Geometry check sheet. Reference: drawing and pictorial views, mm from the part's lowest x, y, z. A direction names the side the tool comes from. Give positions to 0.01 mm unless a question says otherwise; leave off trailing zeros. Loops run counter-clockwise (first coordinate to the right, second up) from the corner with the lowest first, then second, coordinate; pieces in that order, holes last. Notation, with made-up numbers: (-24, 6.5) -> (5, 6.5) arc R22 ccw to (5, 23.5) -> close; hole circle Ø6 at (66, 88). An arc over 180 degrees is marked (long way). One line per item, written item: value. Start each with the question number.
(1) Tool access check on the marked faces 1, 2 and 3. Record the directions out of +Z, -Z, +X, -X, +Y, -Y that give a thin tool (end or side, any length) a straight path to the whole face; none if there is none.
(2) Sectioned sample at C-C, the plane z = 16.5. Record the cut outline in (x, y) (1 decimal).
(3) Scan lines: line 1 along Y through (x, z) = (4, 8.75); line 2 along X through (y, z) = (3.5, 16.5); line 3 along Y through (x, z) = (1.5, 23.25) (1 decimal). Record each from-to range of solid material in increasing order. Write a range as from..to.
(4) Gauge pin test, flat ends, axial feed: pin 1 Ø1 at (x, z) = (1.5, 21) entering from +Y; pin 2 Ø1.5 at (x, z) = (5, 25.5) entering from +Y; pin 3 Ø1 at (x, y) = (6.5, 1) entering from -Z (3 decimals). Record the tip position at first contact, or that the pin passes through.
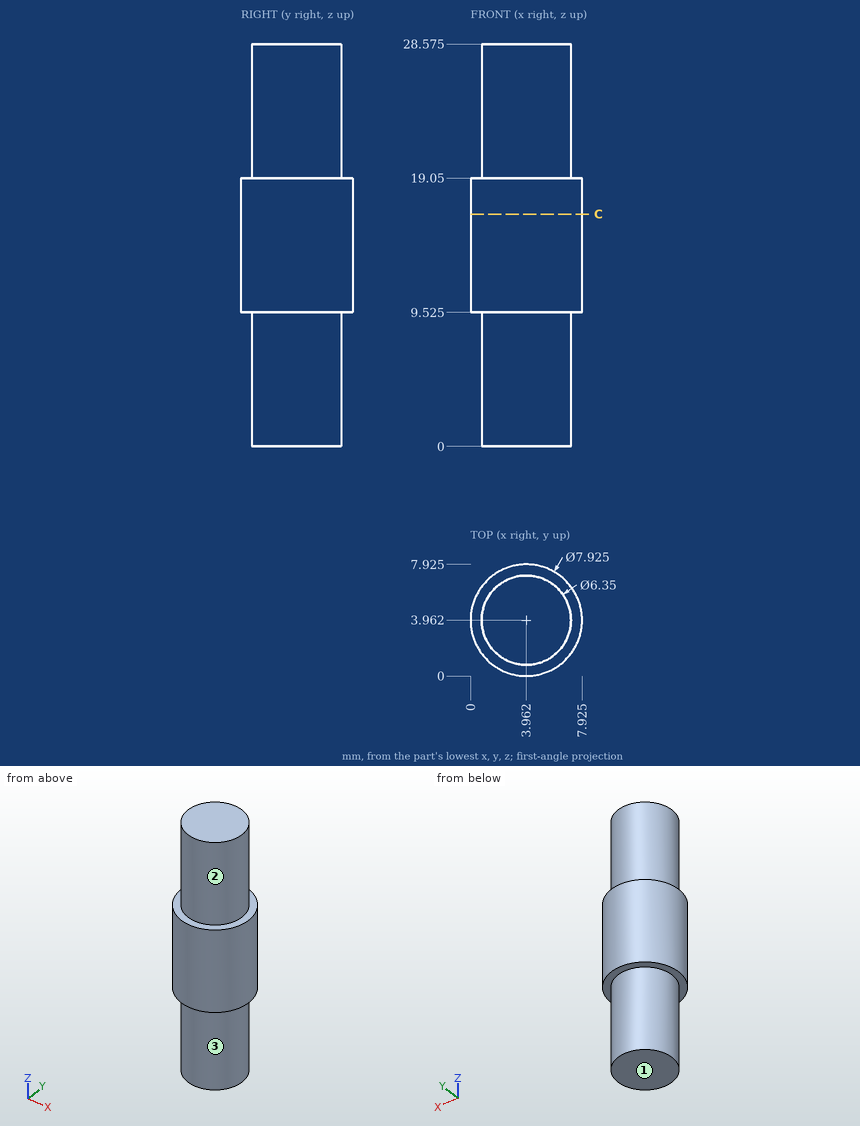
Calculated:
1. face 1: -Z, +X, -X, +Y, -Y
1. face 2: +Z
1. face 3: -Z
2. outline: circle Ø7.9 at (4, 4)
3. line 1: y = 0.79..7.14
3. line 2: x = 0.03..7.9
3. line 3: y = 2..6
4. pin 1: stops at y = 6.46
4. pin 2: stops at y = 7.12
4. pin 3: stops at z = 9.525
